Work out the finished part from the listing and answer in its coordinate system (mm). A direction names the side the tool comes from. Coordinates: 2 decimals unless noted, no trailing zeros. Write each loop counter-clockwise with the first axis right and the second up, starting at its lowest first coordinate (ties: lowest second). Pieces come first, ordered by that corner, then holes. Notation, with made-up numbers: M 86.25,29 L 95.25,29 A34 ccw 95.25,62 Z; hole C 66,-20.75 d4. An arc over 180 degrees is marked long. Use CSV: the item, a comma, the result in double quotes.
from build123d import *

# Parameters (mm, degrees)
EXTRUDE_1_DEPTH        = 13.5
SKETCH_2_W             = 21
SKETCH_2_H             = 6
SKETCH_2_H_2           = 15
CUT_EXTRUDE_1_DEPTH    = 2
FILLET_1_R             = 1
SKETCH_3_R             = 2.1
CUT_EXTRUDE_2_DEPTH    = 58
HOLE_WIZARD_M5_1_D     = 4.2
HOLE_WIZARD_M5_1_DEPTH = 8
HOLE_WIZARD_M5_1_TIP   = 1.2618073


with BuildPart() as part:
    # 草图1 → 凸台-拉伸1 (new, symmetric)
    with BuildSketch(Plane.XY):
        Polygon((0, 0), (0, 29), (17, 29), (17, 19), (11, 19), (11, 9), (17, 9), (17, -9), (11, -9), (11, -19), (17, -19), (17, -29), (0, -29), align=None)
    extrude(amount=EXTRUDE_1_DEPTH, both=True)

    # 草图2 → 切除-拉伸1 (cut)
    with BuildSketch(Plane(origin=(17, 0, 0), x_dir=(0, 0, -1), z_dir=(1, 0, 0))):
        with Locations((0, 24)):
            Rectangle(SKETCH_2_W, SKETCH_2_H)
        Rectangle(SKETCH_2_W, SKETCH_2_H_2)
        with Locations((0, -24)):
            Rectangle(SKETCH_2_W, SKETCH_2_H)
    extrude(amount=-CUT_EXTRUDE_1_DEPTH, mode=Mode.SUBTRACT)

    # 圆角1
    fillet_1_edges = [part.edges().sort_by_distance(p)[0] for p in [
        (16, 27, -10.5),
        (16, 21, -10.5),
        (16, 21, 10.5),
        (16, 27, 10.5),
    ]]
    fillet(fillet_1_edges, radius=FILLET_1_R)

    # 草图3 → 切除-拉伸2 (cut)
    with BuildSketch(Plane(origin=(0, 29, 0), x_dir=(1, 0, 0), z_dir=(0, 1, 0))):
        with Locations(Location((4.4, 0, 0), (0, 0, 180))):
            Circle(SKETCH_3_R)
    extrude(amount=-CUT_EXTRUDE_2_DEPTH, mode=Mode.SUBTRACT)

    # M5 螺纹孔1
    with Locations(Plane(origin=(4.4, 29, 0), x_dir=(0, 0, 1), z_dir=(0, 1, 0))):
        with Locations((0, 0)):
            Hole(HOLE_WIZARD_M5_1_D / 2, depth=HOLE_WIZARD_M5_1_DEPTH)
            with Locations((0, 0, -(HOLE_WIZARD_M5_1_DEPTH + HOLE_WIZARD_M5_1_TIP / 2))):  # 118° drill point
                Cone(0, HOLE_WIZARD_M5_1_D / 2, HOLE_WIZARD_M5_1_TIP, mode=Mode.SUBTRACT)


solid = part.part
Item 1: The part is cut by section B-B (z = 0). Write down the section's boundary in (x, y), then the cut area to 3 significant figures.
Answer:
outline,"M 0,-29 L 2.3,-29 L 2.3,29 L 0,29 Z; M 6.5,-29 L 17,-29 L 17,-27 L 15,-27 L 15,-21 L 17,-21 L 17,-19 L 11,-19 L 11,-9 L 17,-9 L 17,-7.5 L 15,-7.5 L 15,7.5 L 17,7.5 L 17,9 L 11,9 L 11,19 L 17,19 L 17,21 L 15,21 L 15,27 L 17,27 L 17,29 L 6.5,29 Z"
area,"568 mm2"
Item 2: The part is cut by section C-C (x = 4.4). Write down the section's boundary in (y, z).
Answer:
outline,"M -29,-13.5 L 29,-13.5 L 29,-2.1 L -29,-2.1 Z; M -29,2.1 L 29,2.1 L 29,13.5 L -29,13.5 Z"
Item 3: Consider probe 1 along Y at (x, z) = (14.5, -3); probe 2 along X at (y, z) = (8, 0); probe 3 along Z at (x, y) = (4.4, -3). Determine where each line is inside the solid, lowest interval first.
Answer:
probe 1,"y = -29 to -19, -9 to 9, 19 to 29"
probe 2,"x = 0 to 2.3, 6.5 to 17"
probe 3,"z = -13.5 to -2.1, 2.1 to 13.5"
Item 4: The part is cut by section A-A (x = 12.25). Write down the section's boundary in (y, z).
Answer:
outline,"M -29,-13.5 L -19,-13.5 L -19,13.5 L -29,13.5 Z; M -9,-13.5 L 9,-13.5 L 9,13.5 L -9,13.5 Z; M 19,-13.5 L 29,-13.5 L 29,13.5 L 19,13.5 Z"
Item 5: The part is cut by section D-D (y = -2). Write down the section's boundary in (x, z).
Answer:
outline,"M 0,-13.5 L 17,-13.5 L 17,-10.5 L 15,-10.5 L 15,10.5 L 17,10.5 L 17,13.5 L 0,13.5 Z; hole C 4.4,0 d4.2"
Item 6: Given pin 1 (3 mm diameter, centred on y = -16, z = 4, fed in from +X); pin 2 (3 mm diameter, centred on y = 24.5, z = -1, fed in from +X), each flat-ended and moving along its own axis, determine where each tip first touches the part or whether it passes through.
Answer:
pin 1,"stops at x = 11"
pin 2,"stops at x = 15"
Item 7: For a pull along Z with two mould halves and no side action, classify faces 4 (the face through (14, -19, 0)), 5 (the face through (16, 0, -10.5)) as released by +Z, released by -Z, zero draft, split by the parting line, or undercut.
Answer:
face 4,"zero draft"
face 5,"undercut"
Item 8: A tool of negligible diameter and unlimited length cuts with its end or side. For faces 1 (the face through (14, -9, 0)), 2 (the face through (17, 8, 0)), 3 (the face through (15, -24, 0)), from which of +Z, -Z, +X, -X, +Y, -Y can it reach the whole face along a straight path? Write none if from no direction.
Answer:
face 1,"+Z, -Z, +X"
face 2,"+Z, -Z, +X, +Y, -Y"
face 3,"+X"
